The figure shows three views and two pictorial views of one solid part (mm, origin at its lowest corner). Answer the questions. Round coordinates to 2 decimals unless told otherwise and drop trailing zeros. Order: outer loops, then holes, each group sorted by start corner. A loop starts at its lowest first (then second) coordinate and runs counter-clockwise, first axis right, second up. Notation, with made-up numbers: M 84.25,81 L 129.25,81 A18 cw 129.25,89 Z; hole C 0,70.25 d5. An arc over 180 degrees is marked long. Answer as CSV lines item,"result".
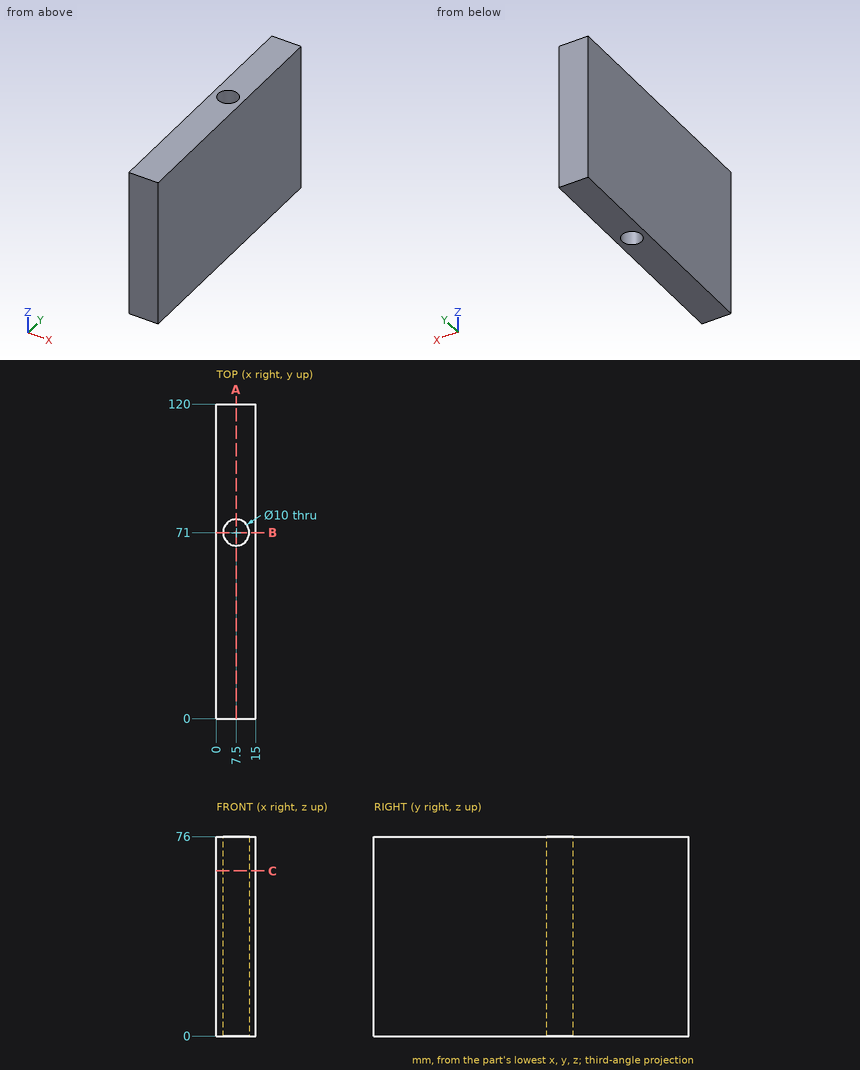
Item 1: Find the intervals of material crossed by probe 1 along Y at (x, z) = (7.5, 33.5); probe 2 along Y at (x, z) = (6, 11.5); probe 3 along X at (y, z) = (73, 13.5), in increasing order. Write a range as [from, to].
Ans:
probe 1,"[0, 66], [76, 120]"
probe 2,"[0, 66.23], [75.77, 120]"
probe 3,"[0, 2.92], [12.08, 15]"
Item 2: A cutting plane is placed at C-C, the plane z = 63. Determine the outline of the cut face in (x, y).
Ans:
outline,"M 0,0 L 15,0 L 15,120 L 0,120 Z; hole C 7.5,71 d10"
Item 3: A cutting plane is placed at A-A, the plane x = 7.5. Determine the outline of the cut face in (y, z).
Ans:
outline,"M 0,0 L 66,0 L 66,76 L 0,76 Z; M 76,0 L 120,0 L 120,76 L 76,76 Z"
Item 4: A flat-ended cylindrical pin translates along its axis: pin 1 (10 mm diameter, centred on y = 73.5, z = 30.5, fed in from -X). Find the tip coordinate at first contact, or state that the pin passes through.
Ans:
pin 1,"x = 0"
Item 5: A cutting plane is placed at B-B, the plane y = 71. Determine the outline of the cut face in (x, z), and give its area (3 significant figures).
Ans:
outline,"M 0,0 L 2.5,0 L 2.5,76 L 0,76 Z; M 12.5,0 L 15,0 L 15,76 L 12.5,76 Z"
area,"380 mm2"
